```python
from build123d import *

# Parameters (mm, degrees)
SKETCH1_R           = 12.5
BOSS_EXTRUDE1_DEPTH = 30
SKETCH2_OUTSIDE_W   = 36.274
SKETCH2_OUTSIDE_H   = 36.274
CUT_EXTRUDE1_DEPTH  = 15
SKETCH3_OUTSIDE_W   = 36.274
SKETCH3_OUTSIDE_H   = 36.274
SKETCH3_OUTSIDE_R   = 8
CUT_EXTRUDE2_DEPTH  = 66.479004269
SKETCH4_R           = 4
BOSS_EXTRUDE2_DEPTH = 8
SKETCH5_OUTSIDE_W   = 29.512
SKETCH5_OUTSIDE_H   = 27.036
SKETCH5_OUTSIDE_R   = 3.25
CUT_EXTRUDE3_DEPTH  = 1.5
SKETCH6_OUTSIDE_W   = 29.512
SKETCH6_OUTSIDE_H   = 27.036
SKETCH6_OUTSIDE_R   = 6
CUT_EXTRUDE4_DEPTH  = 14
SKETCH8_OUTSIDE_W   = 29.512
SKETCH8_OUTSIDE_H   = 27.036
SKETCH8_OUTSIDE_R   = 5.5
CUT_EXTRUDE5_DEPTH  = 1.1
CHAMFER1_SIZE       = 0.2


with BuildPart() as part:
    # Sketch1 → Boss-Extrude1 (new body)
    with BuildSketch(Plane.XY):
        with Locations((0, 50)):
            Circle(SKETCH1_R)
    extrude(amount=BOSS_EXTRUDE1_DEPTH)

    # Sketch2 outside → Cut-Extrude1 (cut)
    with BuildSketch(Plane(origin=(0, 0, 0), x_dir=(-1, 0, 0), z_dir=(0, 0, -1))):
        with Locations((0, 50)):
            Rectangle(SKETCH2_OUTSIDE_W, SKETCH2_OUTSIDE_H)
        Polygon((-4.618802154, 42), (4.618802154, 42), (9.237604307, 50), (4.618802154, 58), (-4.618802154, 58), (-9.237604307, 50), align=None, mode=Mode.SUBTRACT)
    extrude(amount=-CUT_EXTRUDE1_DEPTH, mode=Mode.SUBTRACT)

    # Sketch3 outside → Cut-Extrude2 (cut, through all)
    with BuildSketch(Plane(origin=(0, 0, 15), x_dir=(-1, 0, 0), z_dir=(0, 0, -1))):
        with Locations((0, 50)):
            Rectangle(SKETCH3_OUTSIDE_W, SKETCH3_OUTSIDE_H)
        with Locations((0, 50)):
            Circle(SKETCH3_OUTSIDE_R, mode=Mode.SUBTRACT)
    extrude(amount=-CUT_EXTRUDE2_DEPTH, mode=Mode.SUBTRACT)

    # Sketch4 → Boss-Extrude2 (add)
    with BuildSketch(Plane(origin=(0, 0, 0), x_dir=(-1, 0, 0), z_dir=(0, 0, -1))):
        with Locations(Location((0, 50, 0), (0, 0, 180))):
            Circle(SKETCH4_R)
    extrude(amount=BOSS_EXTRUDE2_DEPTH)

    # Sketch5 outside → Cut-Extrude3 (cut)
    with BuildSketch(Plane(origin=(0, 0, 0), x_dir=(-1, 0, 0), z_dir=(0, 0, -1))):
        with Locations((0, 50)):
            Rectangle(SKETCH5_OUTSIDE_W, SKETCH5_OUTSIDE_H)
        with Locations((0, 50)):
            Circle(SKETCH5_OUTSIDE_R, mode=Mode.SUBTRACT)
    extrude(amount=CUT_EXTRUDE3_DEPTH, mode=Mode.SUBTRACT)

    # Sketch6 outside → Cut-Extrude4 (cut)
    with BuildSketch(Plane.XY.offset(30)):
        with Locations((0, 50)):
            Rectangle(SKETCH6_OUTSIDE_W, SKETCH6_OUTSIDE_H)
        with Locations((0, 50)):
            Circle(SKETCH6_OUTSIDE_R, mode=Mode.SUBTRACT)
    extrude(amount=-CUT_EXTRUDE4_DEPTH, mode=Mode.SUBTRACT)

    # Sketch8 outside → Cut-Extrude5 (cut)
    with BuildSketch(Plane.XY.offset(28)):
        with Locations((0, 50)):
            Rectangle(SKETCH8_OUTSIDE_W, SKETCH8_OUTSIDE_H)
        with Locations((0, 50)):
            Circle(SKETCH8_OUTSIDE_R, mode=Mode.SUBTRACT)
    extrude(amount=CUT_EXTRUDE5_DEPTH, mode=Mode.SUBTRACT)

    # Chamfer1
    chamfer1_edges = [part.edges().sort_by_distance(p)[0] for p in [
        (-4, 50, -8),
        (-6, 50, 30),
    ]]
    chamfer(chamfer1_edges, length=CHAMFER1_SIZE)

    # Sketch10 → Cut-Revolve1 (revolve, cut)
    with BuildSketch(Plane(origin=(0, 50, 0), x_dir=(1, 0, 0), z_dir=(0, 1, 0))):
        Polygon((-9.237604307, 0), (-9.237604307, -2), (-8.082903769, 0), align=None)
        Polygon((-9.237604307, -15), (-9.237604307, -14), (-8.660254038, -15), align=None)
    revolve(axis=Axis((0, 50, -8), (0, 0, 1)), mode=Mode.SUBTRACT)


solid = part.part
```
Input: part model. Units: mm. Frame: model coordinates. A direction names the side the tool comes from. Round coordinates to 2 decimals unless told otherwise and drop trailing zeros. Order: outer loops, then holes, each group sorted by start corner. A loop starts at its lowest first (then second) coordinate and runs counter-clockwise, first axis right, second up. Notation, with made-up numbers: (2, -5.75) - (54, -5.75) arc R27 ccw to (54, 17.25) - close; hole circle Ø7 at (-29.75, 64). An arc over 180 degrees is marked (long way). One line per question, with ' | ' between items. Start each with the question number.
1) Cut plane A-A, the plane z = 13. Return the cut outline in (x, y), then the cut area to 3 significant figures.
2) Pull-direction query (Z, two-part tool) for faces 1 (the flat face through (-6.961, 53.944, 7.395)), 2 (the conical face through (-8.817, 50.016, 14.729)), 3 (the flat face through (3, 45, 29.1)); classes: +Z half, -Z half, draft (parallel to the pull), parting line (faces both ways), or undercut.
3) Set-up query: faces 4 (the cylindrical face through (-1.301, 44.143, 29.455)), 5 (the cylindrical face through (1.846, 53.549, -4.606)), 6 (the flat face through (-4.2, 57, 15)). Return all of +Z, -Z, +X, -X, +Y, -Y with unobstructed straight access to the full face (end or side cutting, diameter ignored); none if empty.
4) Ray query, probe 1 along Z at (x, y) = (-3.75, 50.75); probe 2 along Z at (x, y) = (-6, 49); probe 3 along Z at (x, y) = (0, 54.25). Return the intervals inside material, ascending.
5) Contact query for flat-ended pins moving along their axis: P1, Ø3, axis at x = -3.5, y = 43.5, coming from the +Z side; P2, Ø8, axis at y = 55, z = -1, coming from the +X side; P3, Ø4, axis at y = 56, z = 14.5, coming from the +X side. Output: stop coordinate, or through.
Worked out:
1) outline: (-9.24, 50) - (-4.62, 42) - (4.62, 42) - (9.24, 50) - (4.62, 58) - (-4.62, 58) - close | area: 222 mm^2
2) face 1: draft | face 2: +Z half | face 3: undercut
3) face 4: +Z | face 5: -Z | face 6: +Z, -X, +Y
4) probe 1: z = -7.98 to -1.5, 0 to 30 | probe 2: z = 0 to 16 | probe 3: z = 0 to 30
5) P1: stops at z = 29.92 | P2: stops at x = 8.42 | P3: stops at x = 6.93
